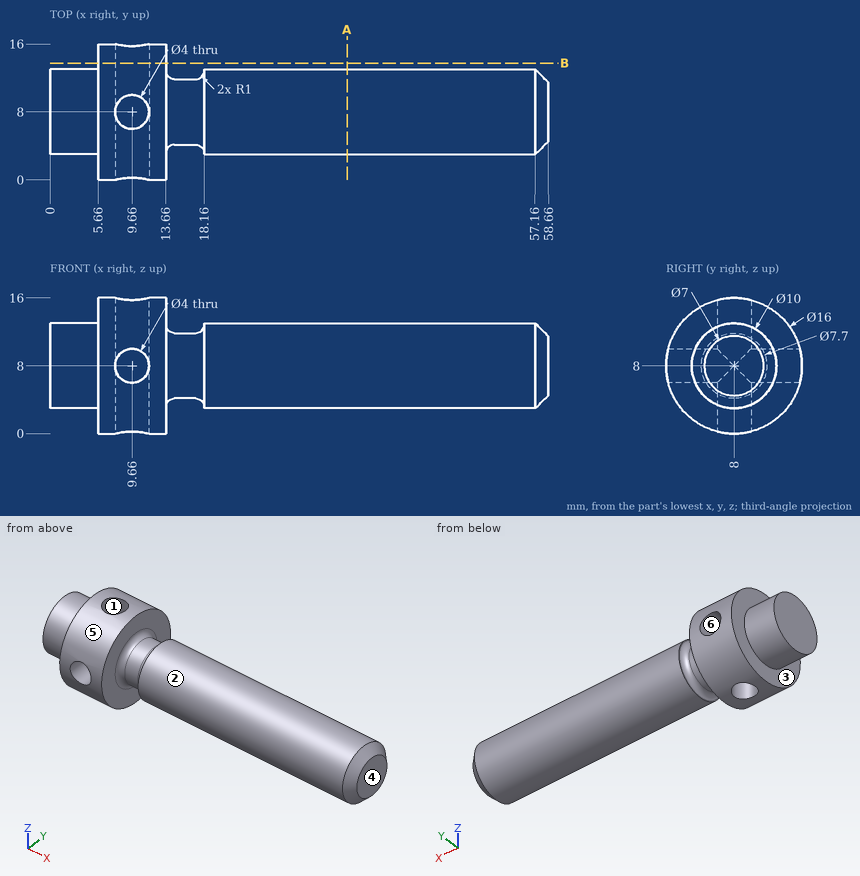
Check sheet for the drawn part. Datum: minimum x, y, z corner. Units: mm. A direction names the side the tool comes from. Round coordinates to 2 decimals unless told otherwise and drop trailing zeros. Loops run counter-clockwise (first coordinate to the right, second up) from the corner with the lowest first, then second, coordinate; pieces in that order, holes last. Notation, with made-up numbers: (-28, -3) - (-24, -3) arc R38 ccw to (-24, 35) - close; hole circle Ø3 at (7.25, 89.5). An arc over 180 degrees is marked (long way). Answer as a JSON object with one key per item and string values. Group by question number.
Q1. Gauge pin test, flat ends, axial feed: P1, Ø3, axis at x = 29, z = 3, coming from the -Y side; P2, Ø5, axis at x = 48.5, y = 7.5, coming from the +Z side; P3, Ø1.5, axis at y = 6, z = 2, coming from the -X side; P4, Ø8, axis at y = 5, z = 9.5, coming from the -X side. Record the tip position at first contact, or that the pin passes through.
Q2. Set-up check for the marked faces 1, 2 and 3: record each of +Z, -Z, +X, -X, +Y, -Y from which the full face is reachable in a straight line by a thin tool's end or side.
Q3. Scan lines: line 1 along X through (y, z) = (3.25, 8) (1 decimal); line 2 along X through (y, z) = (14, 8); line 3 along Y through (x, z) = (30, 6.75). Record each from-to range of solid material in increasing order. Write a range as [from, to].
Q4. Sectioned sample at A-A, the plane x = 35. Enter the section's corners in (y, z).
Q5. Sectioned sample at B-B, the plane y = 13.75. Enter the section's corners in (x, z).
Q6. Mould release check, pull along Z, two halves, no side actions. Record for the marked faces 4, 5 and 6: released by +Z, released by -Z, zero draft, split by the parting line, or undercut.
Solution:
{
 "1": {"P1": "stops at y = 4.43", "P2": "stops at z = 13", "P3": "stops at x = 5.66", "P4": "stops at x = 0"},
 "2": {"face 1": "+Z, -Z", "face 2": "+X", "face 3": "-X"},
 "3": {"line 1": "x = [0, 7.7], [11.7, 13.7], [18.2, 57.4]", "line 2": "x = [5.66, 7.66], [11.66, 13.66]", "line 3": "y = [3.16, 12.84]"},
 "4": {"outline": "circle Ø10 at (8, 8)"},
 "5": {"outline": "(5.66, 2.44) - (13.66, 2.44) - (13.66, 13.56) - (5.66, 13.56) - close; hole circle Ø4 at (9.66, 8)"},
 "6": {"face 4": "zero draft", "face 5": "split by the parting line", "face 6": "undercut"}
}
